Source: CAD feature listing. Evaluate the final solid. Frame: model axes, mm. A direction names the side the tool comes from. Coordinates: 2 decimals unless noted, no trailing zeros. Write each loop counter-clockwise with the first axis right and the second up, starting at its lowest first coordinate (ties: lowest second). Pieces come first, ordered by that corner, then holes. Notation, with made-up numbers: M 18,26 L 68,26 A27 ccw 68,62 Z; hole C 81,20 d7. An arc over 180 degrees is marked long. Write item = value, one per line. Start each with the question number.
1. Section query C-C (y = 4). Output: boundary loops of the cut face in (x, z).
2. Line query: line 1 along Z through (x, y) = (-4.75, -7); line 2 along Y through (x, z) = (1, 7.25); line 3 along X through (y, z) = (-2, 4.5). Output: solid intervals per line, ascending.
3. Section query B-B (y = -9). Output: boundary loops of the cut face in (x, z), then the cut area to 3 significant figures.
4. Access query for faces 1 (the face through (0, 0, -8)), 2 (the face through (-10, 20, 5)), 3 (the face through (0, 22, 0)), 4 (the face through (0, -20, 0)), 5 (the face through (0, 0, 8)). Directions: +Z, -Z, +X, -X, +Y, -Y. A direction counts if a zero-diameter tool reaches every point of the face in a straight line with its end or side. Return the directions, or none.
5. Pin query (flat end, axial travel): pin 1 Ø3 at (x, y) = (-3.5, -12.5) entering from -Z; pin 2 Ø1.5 at (x, z) = (-1, -7.5) entering from -Y; pin 3 Ø2 at (y, z) = (10.5, 6.5) entering from +X. Return the tip coordinate at first contact, or that it passes through.
6. Section query A-A (x = 0). Output: boundary loops of the cut face in (y, z).
```python
from build123d import *
from build123d.topology import SkipClean

# Parameters (mm, degrees)
SKETCH_1_R      = 11
EXTRUDE_1_DEPTH = 20
EXTRUDE_START   = 20
SKETCH_2_W      = 18.439088914
SKETCH_2_H      = 12
EXTRUDE_2_DEPTH = 20
SKETCH_3_R      = 12.5
EXTRUDE_3_DEPTH = 2
CHAMFER_1_SIZE  = 1
CHAMFER_1_SIZE2 = 3


with BuildPart() as part:
    # 草图1 → 凸台-拉伸1 (new body)
    with BuildSketch(Plane(origin=(0, 0, 0), x_dir=(1, 0, 0), z_dir=(0, 1, 0))):
        with Locations(Location((0, 0, 0), (0, 0, 270))):
            Circle(SKETCH_1_R)
    extrude(amount=EXTRUDE_1_DEPTH)

    # 草图2 → 凸台-拉伸2 (add)
    with SkipClean():  # the faces are left unmerged after this step: merging them gives an invalid solid
        with BuildSketch(Plane.XZ.offset(EXTRUDE_START)):
            with BuildLine():
                Line((-9.219544457, -6), (-9.219544457, 6))
                ThreePointArc((-9.219544457, 6), (-11, 0), (-9.219544457, -6))
            make_face()
            Rectangle(SKETCH_2_W, SKETCH_2_H)
            with BuildLine():
                ThreePointArc((11, 0), (10.545496409, 3.129297922), (9.219544457, 6))
                Line((9.219544457, 6), (9.219544457, -6))
                ThreePointArc((9.219544457, -6), (10.545496409, -3.129297922), (11, 0))
            make_face()
        extrude(amount=-EXTRUDE_2_DEPTH)

    # 草图3 → 凸台-拉伸3 (add)
    with SkipClean():  # the faces are left unmerged after this step: merging them gives an invalid solid
        with BuildSketch(Plane(origin=(0, 20, 0), x_dir=(1, 0, 0), z_dir=(0, 1, 0))):
            with Locations(Location((0, 0, 0), (0, 0, 270))):
                Circle(SKETCH_3_R)
        extrude(amount=EXTRUDE_3_DEPTH)

    # 倒角1
    chamfer_1_edges = [part.edges().sort_by_distance(p)[0] for p in [
        (0, 22, -12.5),
    ]]
    chamfer_1_side = [part.faces().sort_by_distance(p)[0] for p in [
        (0, 21, -12.5),
    ]]
    chamfer(chamfer_1_edges, length=CHAMFER_1_SIZE, length2=CHAMFER_1_SIZE2, reference=chamfer_1_side[0])


solid = part.part
```
Results are:
q1.outline = C 0,0 d22
q2.line_1 = -6 to 6
q2.line_2 = 0 to 22
q2.line_3 = -10.04 to 10.04
q3.outline = M -9.22,-6 L 9.22,-6 A11 ccw 9.22,6 L -9.22,6 A11 ccw Z
q3.area = 250 mm^2
q4.face_1 = -Z, +X, -X, -Y
q4.face_2 = -Y
q4.face_3 = +Z, -Z, +X, -X, +Y
q4.face_4 = +Z, -Z, +X, -X, -Y
q4.face_5 = +Z, +X, -X, -Y
q5.pin_1 = -6
q5.pin_2 = 0
q5.pin_3 = 9.53
q6.outline = M -20,-6 L 0,-6 L 0,-11 L 20,-11 L 20,-12.5 L 21,-12.5 L 22,-9.5 L 22,9.5 L 21,12.5 L 20,12.5 L 20,11 L 0,11 L 0,6 L -20,6 Z
